Design review of the part built by this model. Coordinates are the model's own, in mm. A direction names the side the tool comes from. Give positions to 0.01 mm unless a question says otherwise; leave off trailing zeros. Order: outer loops, then holes, each group sorted by start corner. A loop starts at its lowest first (then second) coordinate and runs counter-clockwise, first axis right, second up.
```python
from build123d import *

# Parameters (mm, degrees)
SKETCH1_W             = 300
SKETCH1_H             = 160
BOSS_EXTRUDE1_DEPTH   = 15
CHAMFER1_SIZE         = 3
SKETCH2_R             = 14
CUT_EXTRUDE1_DEPTH    = 171.660481659
M4_TAPPED_HOLE1_D     = 3.3
SKETCH5_R             = 14.5
CUT_EXTRUDE2_DEPTH    = 171.660481659
M6_TAPPED_HOLE1_D     = 5
M5_TAPPED_HOLE2_D     = 4.2
M5_TAPPED_HOLE2_DEPTH = 14
M5_TAPPED_HOLE2_TIP   = 1.2618073
SKETCH17_W            = 220
SKETCH17_H            = 40
CUT_EXTRUDE6_DEPTH    = 171.660481755
M6_TAPPED_HOLE2_D     = 5
SKETCH20_R            = 20
CUT_EXTRUDE7_DEPTH    = 171.660481755
CHAMFER2_SIZE         = 3
FILLET1_R             = 5


with BuildPart() as part:
    # Sketch1 → Boss-Extrude1 (new body)
    with BuildSketch(Plane(origin=(0, 0, 0), x_dir=(1, 0, 0), z_dir=(0, 1, 0))):
        Rectangle(SKETCH1_W, SKETCH1_H)
    extrude(amount=BOSS_EXTRUDE1_DEPTH)

    # Chamfer1
    chamfer1_edges = [part.edges().sort_by_distance(p)[0] for p in [
        (-150, 7.5, -80),
        (150, 7.5, -80),
        (150, 7.5, 80),
        (-150, 7.5, 80),
    ]]
    chamfer(chamfer1_edges, length=CHAMFER1_SIZE)

    # Sketch2 → Cut-Extrude1 (cut, through all)
    with BuildSketch(Plane(origin=(0, 15, 0), x_dir=(1, 0, 0), z_dir=(0, 1, 0))):
        with Locations(Location((130, -50, 0), (0, 0, 270))):
            Circle(SKETCH2_R)
        with Locations(Location((130, 52, 0), (0, 0, 90))):
            Circle(SKETCH2_R)
    extrude(amount=-CUT_EXTRUDE1_DEPTH, mode=Mode.SUBTRACT)

    # M4 Tapped Hole1 (through all)
    with Locations(Plane(origin=(0, 15, 0), x_dir=(-1, 0, 0), z_dir=(0, 1, 0))):
        with Locations((-141, 34.5), (-119, -67.5), (-141, -67.5), (-119, -36.5), (-141, -36.5), (-119, 34.5), (-119, 65.5), (-141, 65.5)):
            Hole(M4_TAPPED_HOLE1_D / 2)

    # Sketch5 → Cut-Extrude2 (cut, through all)
    with BuildSketch(Plane(origin=(0, 15, 0), x_dir=(1, 0, 0), z_dir=(0, 1, 0))):
        with Locations(Location((130, 1, 0), (0, 0, 270))):
            Circle(SKETCH5_R)
    extrude(amount=-CUT_EXTRUDE2_DEPTH, mode=Mode.SUBTRACT)

    # M6 Tapped Hole1 (through all)
    with Locations(Plane(origin=(0, 15, 0), x_dir=(-1, 0, 0), z_dir=(0, 1, 0))):
        with Locations((-130, -20), (-130, 18)):
            Hole(M6_TAPPED_HOLE1_D / 2)

    # M5 Tapped Hole2
    with Locations(Plane(origin=(150, 0, 0), x_dir=(0, 0, -1), z_dir=(1, 0, 0))):
        with Locations((-38.5, 7.5), (-61.5, 7.5)):
            Hole(M5_TAPPED_HOLE2_D / 2, depth=M5_TAPPED_HOLE2_DEPTH)
            with Locations((0, 0, -(M5_TAPPED_HOLE2_DEPTH + M5_TAPPED_HOLE2_TIP / 2))):  # 118° drill point
                Cone(0, M5_TAPPED_HOLE2_D / 2, M5_TAPPED_HOLE2_TIP, mode=Mode.SUBTRACT)

    # Sketch17 → Cut-Extrude6 (cut, through all)
    with BuildSketch(Plane(origin=(0, 15, 0), x_dir=(1, 0, 0), z_dir=(0, 1, 0))):
        with Locations((-40, 60)):
            Rectangle(SKETCH17_W, SKETCH17_H)
        with Locations((-40, -60)):
            Rectangle(SKETCH17_W, SKETCH17_H)
    extrude(amount=-CUT_EXTRUDE6_DEPTH, mode=Mode.SUBTRACT)

    # M6 Tapped Hole2 (through all)
    with Locations(Plane(origin=(0, 15, 0), x_dir=(1, 0, 0), z_dir=(0, 1, 0))):
        with Locations((-130, 25), (-130, -25), (20, -25), (20, 25)):
            Hole(M6_TAPPED_HOLE2_D / 2)

    # Sketch20 → Cut-Extrude7 (cut, through all)
    with BuildSketch(Plane(origin=(0, 15, 0), x_dir=(1, 0, 0), z_dir=(0, 1, 0))):
        with Locations(Location((-55, 0, 0), (0, 0, 270))):
            Circle(SKETCH20_R)
    extrude(amount=-CUT_EXTRUDE7_DEPTH, mode=Mode.SUBTRACT)

    # Chamfer2
    chamfer2_edges = [part.edges().sort_by_distance(p)[0] for p in [
        (70, 7.5, -80),
        (-150, 7.5, -40),
        (-150, 7.5, 40),
        (70, 7.5, 80),
    ]]
    chamfer(chamfer2_edges, length=CHAMFER2_SIZE)

    # Fillet1
    fillet1_edges = [part.edges().sort_by_distance(p)[0] for p in [
        (70, 7.5, -40),
        (70, 7.5, 40),
    ]]
    fillet(fillet1_edges, radius=FILLET1_R)


solid = part.part
```
1. Machinability: for faces 5 (the face through (70, 8, -61)), 6 (the face through (-2, 0, -1)), 7 (the face through (70, 8, 61)), which of the approach directions +Z, -Z, +X, -X, +Y, -Y give a long, thin tool a straight path to every point of the face, cutting with its end or side? Answer none if there is none.
Recorded:
face 5: -Z, -X, +Y, -Y
face 6: +Z, -Z, +X, -X, -Y
face 7: +Z, -X, +Y, -Y
2. Take a section at A-A (y = 2.5). State how many separate pieces and enclosed holes the cut face has, then the cut area to 3 significant figures.
Recorded:
separate pieces: 1
enclosed holes: 18
area: 27,000 mm2
3. Take a section at B-B (z = -2). State the section outline as (x, y) points.
Recorded:
outline: (-150, 0) - (-74.9, 0) - (-74.9, 15) - (-150, 15) - close; (-35.1, 0) - (115.53, 0) - (115.53, 15) - (-35.1, 15) - close; (144.47, 0) - (150, 0) - (150, 15) - (144.47, 15) - close
4. For line 1 along Z through (x, y) = (-130, 11); line 2 along X through (y, z) = (4, 25); line 3 along X through (y, z) = (3.25, -67.5), list the stretches that pass through material, from the lowest coordinate up.
Recorded:
line 1: z = -40 to -27.5, -22.5 to 22.5, 27.5 to 40
line 2: x = -150 to -132.5, -127.5 to 17.5, 22.5 to 150
line 3: x = 70 to 117.35, 120.65 to 139.35, 142.65 to 150
5. Draft analysis for pull direction Z (two halves, no side actions). For faces 1 (the face through (-42, 8, -40)), 2 (the face through (116.12, 7.6, -50.18)), 3 (the face through (115.845, 7.605, -4.143)), 4 (the face through (-2, 15, -1)), state which applies: pulls with the +Z half, pulls with the -Z half, needs draft (parallel to the pull), parting line crosses it, or undercut.
Recorded:
face 1: pulls with the -Z half
face 2: undercut
face 3: undercut
face 4: needs draft
6. Take a section at C-C (x = 46). State the section outline as (y, z) points.
Recorded:
outline: (0, -40) - (15, -40) - (15, 40) - (0, 40) - close
7. For pin 1 (1.5 mm diameter, centred on x = -37.5, y = 4.5, fed in from -Z); pin 2 (7.5 mm diameter, centred on y = 8, z = -58.5, fed in from -X); pin 3 (1.5 mm diameter, centred on x = -80, y = 6.5, fed in from +Z), all flat-tipped, find the tip position at first contact; note any pin that passes through.
Recorded:
pin 1: stops at z = -40
pin 2: stops at x = 70
pin 3: stops at z = 40
